```python
from build123d import *

# Parameters (mm, degrees)
BASE_PLATE_SKETCH_W          = 110
BASE_PLATE_SKETCH_H          = 45
BASE_PLATE_DEPTH             = 12
SECOND_BLOCK_SKETCH_W        = 110
SECOND_BLOCK_SKETCH_H        = 50
SECOND_BLOCK_DEPTH           = 12
LEG_PROFILE_BOSS_DEPTH       = 23
SEMICIRCULAR_START           = -12
SEMICIRCULAR_NOTCH_CUT_DEPTH = 12


with BuildPart() as part:
    # Base Plate Sketch → Base Plate (new body)
    with BuildSketch(Plane.XY):
        with Locations((55, 22.5)):
            Rectangle(BASE_PLATE_SKETCH_W, BASE_PLATE_SKETCH_H)
    extrude(amount=BASE_PLATE_DEPTH)

    # Second Block Sketch → Second Block (add)
    with BuildSketch(Plane(origin=(0, 45, 0), x_dir=(1, 0, 0), z_dir=(0, 1, 0))):
        with Locations((55, -37)):
            Rectangle(SECOND_BLOCK_SKETCH_W, SECOND_BLOCK_SKETCH_H)
    extrude(amount=-SECOND_BLOCK_DEPTH)

    # Leg Profile Sketch → Leg Profile Boss (add)
    with BuildSketch(Plane.XZ.offset(-33)):
        with BuildLine():
            Line((80, 62), (80, 52))
            Line((80, 52), (77, 52))
            Line((77, 52), (66, 12))
            Line((66, 12), (55, 12))
            Line((55, 12), (44, 12))
            Line((44, 12), (33, 52))
            Line((33, 52), (30, 52))
            Line((30, 52), (30, 62))
            Line((30, 62), (40, 62))
            ThreePointArc((40, 62), (55, 47), (70, 62))
            Line((70, 62), (80, 62))
        make_face()
    extrude(amount=LEG_PROFILE_BOSS_DEPTH)

    # Semicircular Notch Sketch → Semicircular Notch Cut (cut)
    with BuildSketch(Plane.XZ.offset(-33).offset(SEMICIRCULAR_START)):
        with BuildLine():
            Line((40, 62), (70, 62))
            ThreePointArc((70, 62), (55, 47), (40, 62))
        make_face()
    extrude(amount=SEMICIRCULAR_NOTCH_CUT_DEPTH, mode=Mode.SUBTRACT)


solid = part.part
```
Model file for the job. Use its own axes, mm. A direction names the side the tool comes from. Give positions to 0.01 mm unless a question says otherwise; leave off trailing zeros. Write each loop counter-clockwise with the first axis right and the second up, starting at its lowest first coordinate (ties: lowest second). Pieces come first, ordered by that corner, then holes. Notation, with made-up numbers: (15, 25) -> (30, 25) arc R9 cw to (30, 30) -> close; hole circle Ø3 at (23.5, -17). An arc over 180 degrees is marked (long way). Use CSV: the item, a comma, the result in double quotes. Start each with the question number.
1) Cut at B-B on y = 24. List the corners of the cut face in (x, z).
2) Tool access for faces 1 (the flat face through (30, 22, 57)), 2 (the flat face through (38.577, 21.661, 31.72)), 3 (the flat face through (71.577, 21.661, 32.28)), 4 (the flat face through (110, 38, 18)), 5 (the flat face through (55, 10, 37)): list every direction of +Z, -Z, +X, -X, +Y, -Y with a clear straight run to the whole face (end or side of a thin tool).
3) Cut at C-C on x = 55. List the corners of the cut face in (y, z), plus the area to 4 significant figures.
4) Cut at A-A on z = 42. List the corners of the cut face in (x, y).
5) Cut at D-D on z = 24. List the corners of the cut face in (x, y), plus the area to 3 significant figures.
6) Pin check, flat tips, straight feed: P1, Ø2.5, axis at x = 31.5, y = 18, coming from the -Z side; P2, Ø3, axis at y = 18.5, z = 58.5, coming from the +X side; P3, Ø22, axis at x = 21.5, z = 37, coming from the -Y side; P4, Ø5, axis at x = 50.5, z = 42.5, coming from the -Y side. Stop position of each tip, or through.
7) Drill centre lines: L1, parallel to Y at x = 93.5, z = 50.5; L2, parallel to Z at x = 80.5, y = 17; L3, parallel to X at y = 19, z = 44. Where is each one in solid material? Low to high.
8) Two-plate mould, pull along Z, no slides. Class faces 6 (the flat face through (24, 36, 62)), 7 (the flat face through (54, 23, 0)), 8 (the flat face through (54, 9, 12)), 9 (the flat face through (80, 22, 57)): released by +Z, released by -Z, zero draft, split by the parting line, or undercut.
Final values:
1,outline,"(0, 0) -> (110, 0) -> (110, 12) -> (66, 12) -> (77, 52) -> (80, 52) -> (80, 62) -> (70, 62) arc R15 cw to (40, 62) -> (30, 62) -> (30, 52) -> (33, 52) -> (44, 12) -> (0, 12) -> close"
2,face 1,"+Z, -X, -Y"
2,face 2,"-X, -Y"
2,face 3,"+X, -Y"
2,face 4,"+Z, -Z, +X, +Y, -Y"
2,face 5,"+Z, +X, -X, -Y"
3,outline,"(0, 0) -> (45, 0) -> (45, 47) -> (10, 47) -> (10, 12) -> (0, 12) -> close"
3,area,"1,765 mm2"
4,outline,"(0, 33) -> (35.75, 33) -> (35.75, 10) -> (74.25, 10) -> (74.25, 33) -> (110, 33) -> (110, 45) -> (0, 45) -> close"
5,outline,"(0, 33) -> (40.7, 33) -> (40.7, 10) -> (69.3, 10) -> (69.3, 33) -> (110, 33) -> (110, 45) -> (0, 45) -> close"
5,area,"1,980 mm2"
6,P1,"stops at z = 0"
6,P2,"stops at x = 80"
6,P3,"stops at y = 33"
6,P4,"stops at y = 10"
7,L1,"y = 33 to 45"
7,L2,"z = 0 to 12"
7,L3,"x = 35.2 to 74.8"
8,face 6,"released by +Z"
8,face 7,"released by -Z"
8,face 8,"undercut"
8,face 9,"zero draft"
